Design review of the part built by this model. Coordinates are the model's own, in mm. Face numbers are marked on the shaded views. A direction names the side the tool comes from. Give positions to 0.01 mm unless a question says otherwise; leave off trailing zeros. Loops run counter-clockwise (first coordinate to the right, second up) from the corner with the lowest first, then second, coordinate; pieces in that order, holes last. Notation, with made-up numbers: (85, 28.25) -> (123, 28.25) arc R25 ccw to (123, 67.25) -> close; hole circle Ø1 at (74.25, 89.5). An arc over 180 degrees is marked (long way). Use a Markdown table: item, result. Add a question column.
1. Draft analysis for pull direction X (two halves, no side actions). For the marked faces 1, 2 and 3, state which applies: pulls with the +X half, pulls with the -X half, needs draft (parallel to the pull), parting line crosses it, or undercut.
2. Add section A-A (y = 0). State the section outline as (x, z) points, and give its area (3 significant figures).
3. To check wall thickness, follow line 1 (Y direction, x = 0, z = 42); line 2 (Z direction, x = 47.5, y = -25); line 3 (X direction, y = 38, z = 52). State the ranges of each line that lie inside material, in increasing order.
4. Add section C-C (z = 27.5). State the section outline as (x, y) points.
5. For pin 1 Ø5 at (x, y) = (5.5, -53.5) entering from +Z; pin 2 Ø8 at (x, z) = (13, 103) entering from -Y; pin 3 Ø5 at (x, z) = (39.5, 23.5) entering from -Y, all flat-tipped, find the tip position at first contact; note any pin that passes through.
6. For the marked faces 4 and 5, list the 3-axis set-ups (+Z, -Z, +X, -X, +Y, -Y) from which the entire face can be reached by the end or side of a thin tool; tool diameter is ignored.
7. Add section D-D (z = 184). State the section outline as (x, y) points, and give its area (3 significant figures).
```python
from build123d import *

# Parameters (mm, degrees)
SKETCH_1_R          = 74.75
EXTRUDE_1_DEPTH     = 70
SKETCH_2_R          = 16.25
CUT_EXTRUDE_1_DEPTH = 68
SKETCH_3_R          = 30
EXTRUDE_2_DEPTH     = 140


with BuildPart() as part:
    # 草图1 → 凸台-拉伸1 (new body)
    with BuildSketch(Plane.XY):
        Circle(SKETCH_1_R)
    extrude(amount=EXTRUDE_1_DEPTH)

    # 草图2 → 切除-拉伸1 (cut)
    with BuildSketch(Plane(origin=(0, 0, 0), x_dir=(-1, 0, 0), z_dir=(0, 0, -1))):
        Circle(SKETCH_2_R)
    extrude(amount=-CUT_EXTRUDE_1_DEPTH, mode=Mode.SUBTRACT)

    # 草图3 → 凸台-拉伸2 (add)
    with BuildSketch(Plane.XY.offset(70)):
        Circle(SKETCH_3_R)
    extrude(amount=EXTRUDE_2_DEPTH)


solid = part.part
```
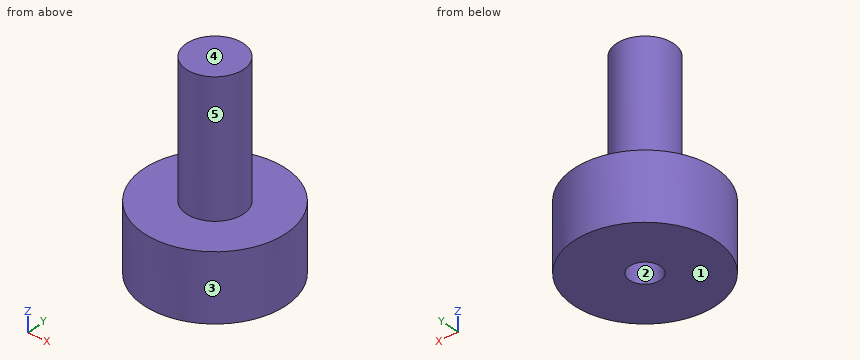
Taken from the geometry:
| question | item | result |
|---|---|---|
| 1 | face 1 | needs draft |
| 1 | face 2 | undercut |
| 1 | face 3 | parting line crosses it |
| 2 | outline | (-74.75, 0) -> (-16.25, 0) -> (-16.25, 68) -> (16.25, 68) -> (16.25, 0) -> (74.75, 0) -> (74.75, 70) -> (30, 70) -> (30, 210) -> (-30, 210) -> (-30, 70) -> (-74.75, 70) -> close |
| 2 | area | 16,700 mm^2 |
| 3 | line 1 | y = -74.75 to -16.25, 16.25 to 74.75 |
| 3 | line 2 | z = 0 to 70 |
| 3 | line 3 | x = -64.37 to 64.37 |
| 4 | outline | circle Ø149.5 at (0, 0); hole circle Ø32.5 at (0, 0) |
| 5 | pin 1 | stops at z = 70 |
| 5 | pin 2 | stops at y = -28.62 |
| 5 | pin 3 | stops at y = -64.95 |
| 6 | face 4 | +Z, +X, -X, +Y, -Y |
| 6 | face 5 | +Z |
| 7 | outline | circle Ø60 at (0, 0) |
| 7 | area | 2,830 mm^2 |
